CAD build for the part. Positions are in the model's coordinates, mm. Coordinates: 2 decimals unless noted, no trailing zeros. Order: outer loops, then holes, each group sorted by start corner. A loop starts at its lowest first (then second) coordinate and runs counter-clockwise, first axis right, second up. Notation, with made-up numbers: (41.5, 37.5) - (80.5, 37.5) arc R29 ccw to (80.5, 60.5) - close; hole circle Ø4 at (39, 37). An arc over 180 degrees is marked (long way). Return JSON: item names as keys, results as strings.
from build123d import *

# Parameters (mm, degrees)
BOSS_EXTRUDE1_DEPTH     = 2334
CUT_EXTRUDE4_DEPTH      = 2337.098456829
CUT_EXTRUDE4_DEPTH_BACK = 10


with BuildPart() as part:
    # Sketch1 → Boss-Extrude1 (new body)
    with BuildSketch(Plane.XY):
        with BuildLine():
            Line((0, 70), (0, 0))
            Line((0, 0), (70, 0))
            Line((70, 0), (70, 5))
            ThreePointArc((70, 5), (69.121320344, 7.121320344), (67, 8))
            Line((67, 8), (16, 8))
            ThreePointArc((16, 8), (10.343145751, 10.343145751), (8, 16))
            Line((8, 16), (8, 67))
            ThreePointArc((8, 67), (7.121320344, 69.121320344), (5, 70))
            Line((5, 70), (0, 70))
        make_face()
    extrude(amount=BOSS_EXTRUDE1_DEPTH)

    # Sketch3 → Cut-Extrude4 (cut, two sides: drawn at the far end of the back side and taken through both)
    with BuildSketch(Plane(origin=(0, 0, 0), x_dir=(0, 0, -1), z_dir=(0.7071067811865488, 0.7071067811865464, 0)).offset(-CUT_EXTRUDE4_DEPTH_BACK)):
        Polygon((0, -49.497474683), (-69.317009791, 49.497474683), (0, 49.497474683), align=None)
        Polygon((-2334, -49.497474683), (-2334, 49.497474683), (-2264.682990209, 49.497474683), align=None)
    extrude(amount=CUT_EXTRUDE4_DEPTH + CUT_EXTRUDE4_DEPTH_BACK, mode=Mode.SUBTRACT)


solid = part.part
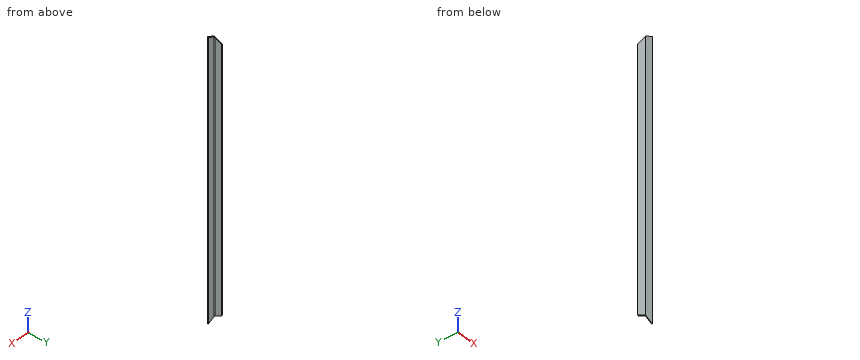
Item 1: Band-saw the part on A-A, the plane z = 1575. List the corners of the cut face in (x, y), then the cut area to 3 significant figures.
Findings below:
{"outline": "(0, 0) - (70, 0) - (70, 5) arc R3 ccw to (67, 8) - (16, 8) arc R8 cw to (8, 16) - (8, 67) arc R3 ccw to (5, 70) - (0, 70) - close", "area": "1,070 mm²"}
Item 2: Drop flat-ended pins along their axis: P1, Ø12, axis at x = 49.5, y = 12, coming from the +Z side; P2, Ø1.5, axis at x = 33.5, z = 1022, coming from the +Y side; P3, Ø2, axis at y = 42.5, z = 714, coming from the +X side. Give the stop position or say it passes through.
Findings below:
{"P1": "stops at z = 2322.11", "P2": "stops at y = 8", "P3": "stops at x = 8"}
Item 3: Band-saw the part on C-C, the plane y = 30.5. List the corners of the cut face in (x, z).
Findings below:
{"outline": "(0, 49.76) - (8, 45.8) - (8, 2288.2) - (0, 2284.24) - close"}
Item 4: Wall check: L1, parallel to Y at x = 33, z = 600; L2, parallel to Y at x = 13.5, z = 831. Give the ranges that are in metal, low to high. Write a range as [from, to].
Findings below:
{"L1": "y = [0, 8]", "L2": "y = [0, 8.4]"}
Item 5: Band-saw the part on B-B, the plane x = 28. List the corners of the cut face in (y, z).
Findings below:
{"outline": "(0, 20.8) - (8, 24.76) - (8, 2309.24) - (0, 2313.2) - close"}
